Build history of the part. All positions in model axes, mm. Face numbers are marked on the shaded views. Give positions to 0.01 mm unless a question says otherwise; leave off trailing zeros. Loops run counter-clockwise (first coordinate to the right, second up) from the corner with the lowest first, then second, coordinate; pieces in that order, holes last. Notation, with made-up numbers: (75.25, 39) - (80.25, 39) arc R29 ccw to (80.25, 64) - close; hole circle Ø4 at (-26.5, 65.25). An arc over 180 degrees is marked (long way). Return JSON: item names as keys, results as strings. Group by question number.
1) Mould opens along X. For the marked faces 1, 2 and 3 say: released by +X, released by -X, zero draft, split by the parting line, or undercut.
2) Drop flat-ended pins along their axis: pin 1 (6 mm diameter, centred on y = 25, z = 16.5, fed in from -X); pin 2 (3 mm diameter, centred on y = -18, z = 19, fed in from +X); pin 3 (1.5 mm diameter, centred on x = -35, z = 8.5, fed in from -Y). Give the stop position or say it passes through.
3) Slice it at A-A (y = 0). List the corners of the cut face in (x, z).
4) Drill centre lines: probe 1 along Y at (x, z) = (0, 7); probe 2 along Y at (x, z) = (32, 5.5). Where is each one in solid material? Low to high. Write a range as from..to.
5) Slice it at C-C (z = 17.75). List the corners of the cut face in (x, y).
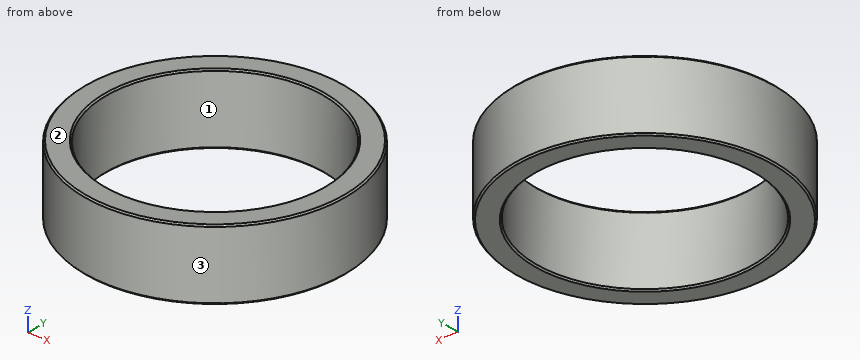
```python
from build123d import *

# Parameters (mm, degrees)
SKETCH1_R           = 45
SKETCH1_R_2         = 37.5
BOSS_EXTRUDE1_DEPTH = 24
CHAMFER1_SIZE       = 0.5


with BuildPart() as part:
    # Sketch1 → Boss-Extrude1 (new body)
    with BuildSketch(Plane.XY):
        Circle(SKETCH1_R)
        Circle(SKETCH1_R_2, mode=Mode.SUBTRACT)
    extrude(amount=BOSS_EXTRUDE1_DEPTH)

    # Chamfer1
    chamfer1_edges = [part.edges().sort_by_distance(p)[0] for p in [
        (-45, 0, 0),
        (-45, 0, 24),
        (-37.5, 0, 0),
        (-37.5, 0, 24),
    ]]
    chamfer(chamfer1_edges, length=CHAMFER1_SIZE)


solid = part.part
```
Results:
{
 "1": {"face 1": "undercut", "face 2": "zero draft", "face 3": "split by the parting line"},
 "2": {"pin 1": "x = -39.26", "pin 2": "x = 41.87", "pin 3": "y = -29.19"},
 "3": {"outline": "(-45, 0.5) - (-44.5, 0) - (-38, 0) - (-37.5, 0.5) - (-37.5, 23.5) - (-38, 24) - (-44.5, 24) - (-45, 23.5) - close; (37.5, 0.5) - (38, 0) - (44.5, 0) - (45, 0.5) - (45, 23.5) - (44.5, 24) - (38, 24) - (37.5, 23.5) - close"},
 "4": {"probe 1": "-45..-37.5, 37.5..45", "probe 2": "-31.64..-19.55, 19.55..31.64"},
 "5": {"outline": "circle Ø90 at (0, 0); hole circle Ø75 at (0, 0)"}
}
